Design review of the part built by this model. Coordinates are the model's own, in mm. A direction names the side the tool comes from. Give positions to 0.01 mm unless a question says otherwise; leave off trailing zeros. Order: outer loops, then holes, each group sorted by start corner. A loop starts at its lowest first (then second) coordinate and runs counter-clockwise, first axis right, second up. Notation, with made-up numbers: (-0.75, 56) -> (33.25, 56) arc R9 cw to (33.25, 61) -> close; hole circle Ø8 at (-6, 39.25). An arc over 180 degrees is marked (long way). Use a Markdown table: item, result. Add a question column.
```python
from build123d import *

# Parameters (mm, degrees)
SKETCH_1_W                = 144
SKETCH_1_H                = 35
EXTRUDE_1_DEPTH           = 5
HOLE_WIZARD_1_D           = 4.5
HOLE_WIZARD_1_CSINK_D     = 8.6
HOLE_WIZARD_1_CSINK_ANGLE = 90
SKETCH_4_W                = 100
SKETCH_4_H                = 15
CUT_EXTRUDE_1_DEPTH       = 75.264729179
CHAMFER_1_SIZE            = 3
FILLET_1_R                = 5


with BuildPart() as part:
    # 草图1 → 凸台-拉伸1 (new body)
    with BuildSketch(Plane.XY):
        Rectangle(SKETCH_1_W, SKETCH_1_H)
    extrude(amount=EXTRUDE_1_DEPTH)

    # 打孔尺寸根据十字槽沉头木螺钉的类型1 (through all)
    with Locations(Plane.XY.offset(5)):
        with Locations((-65.75, 7.5), (-65.75, -7.5), (65.75, 7.5), (65.75, -7.5)):
            CounterSinkHole(HOLE_WIZARD_1_D / 2, HOLE_WIZARD_1_CSINK_D / 2, counter_sink_angle=HOLE_WIZARD_1_CSINK_ANGLE)

    # 草图4 → 切除-拉伸1 (cut, through all)
    with BuildSketch(Plane.XY.offset(5)):
        with Locations((0, 10)):
            Rectangle(SKETCH_4_W, SKETCH_4_H)
    extrude(amount=-CUT_EXTRUDE_1_DEPTH, mode=Mode.SUBTRACT)

    # 倒角1
    chamfer_1_edges = [part.edges().sort_by_distance(p)[0] for p in [
        (-50, 17.5, 2.5),
        (50, 17.5, 2.5),
        (72, -17.5, 2.5),
        (-72, -17.5, 2.5),
        (-72, 17.5, 2.5),
        (72, 17.5, 2.5),
    ]]
    chamfer(chamfer_1_edges, length=CHAMFER_1_SIZE)

    # 圆角1
    fillet_1_edges = [part.edges().sort_by_distance(p)[0] for p in [
        (-50, 2.5, 2.5),
        (50, 2.5, 2.5),
    ]]
    fillet(fillet_1_edges, radius=FILLET_1_R)


solid = part.part
```
1) Machinability: for faces 4 (the flat face through (-51.5, 16, 2.5)), 5 (the flat face through (70.5, 16, 2.5)), which of the approach directions +Z, -Z, +X, -X, +Y, -Y give a long, thin tool a straight path to every point of the face, cutting with its end or side? Answer none if there is none.
2) Add section D-D (x = -25). Give the boundary of the cut face in (y, z).
3) Insertion check: pin 1 (2 mm diameter, centred on x = 20.5, z = 4.5, fed in from +Y). The pin has a flat end and moves straight along its axis. Give the tip position at first contact, or say it passes through.
4) Add section C-C (z = 4.1). Give the boundary of the cut face in (x, y).
5) Add section A-A (x = -65.75). Give the boundary of the cut face in (y, z).
6) Add section B-B (y = -7.5). Give the boundary of the cut face in (x, z), then the cut area to 3 significant figures.
7) The part is to be moulded in two halves that separate along X. For faces 1 (the flat face through (70.5, -16, 2.5)), 2 (the flat face through (-50, 11, 3)), 3 (the flat face through (-70.5, -16, 2.5)), say which applies: +X half, -X half, draft (parallel to the pull), parting line (faces both ways), or undercut.
8) For L1, parallel to Y at x = 65.75, z = 1.85; L2, parallel to X at y = 7.5, z = 2.2; L3, parallel to X at y = -7.5, z = 2.25, list the stretches that pass through material, from the lowest coordinate up. Write a range as [from, to].
Worked answers:
| question | item | result |
|---|---|---|
| 1 | face 4 | +Z, -Z, +Y |
| 1 | face 5 | +Z, -Z, +X, +Y |
| 2 | outline | (-17.5, 0) -> (2.5, 0) -> (2.5, 5) -> (-17.5, 5) -> close |
| 3 | pin 1 | y = 2.5 |
| 4 | outline | (-72, -14.5) -> (-69, -17.5) -> (69, -17.5) -> (72, -14.5) -> (72, 14.5) -> (69, 17.5) -> (53, 17.5) -> (50, 14.5) -> (50, 7.5) arc R5 cw to (45, 2.5) -> (-45, 2.5) arc R5 cw to (-50, 7.5) -> (-50, 14.5) -> (-53, 17.5) -> (-69, 17.5) -> (-72, 14.5) -> close; hole circle Ø6.8 at (-65.75, -7.5); hole circle Ø6.8 at (-65.75, 7.5); hole circle Ø6.8 at (65.75, -7.5); hole circle Ø6.8 at (65.75, 7.5) |
| 5 | outline | (-17.5, 0) -> (-9.75, 0) -> (-9.75, 2.95) -> (-11.8, 5) -> (-17.5, 5) -> close; (-5.25, 0) -> (5.25, 0) -> (5.25, 2.95) -> (3.2, 5) -> (-3.2, 5) -> (-5.25, 2.95) -> close; (9.75, 0) -> (17.5, 0) -> (17.5, 5) -> (11.8, 5) -> (9.75, 2.95) -> close |
| 6 | outline | (-72, 0) -> (-68, 0) -> (-68, 2.95) -> (-70.05, 5) -> (-72, 5) -> close; (-63.5, 0) -> (63.5, 0) -> (63.5, 2.95) -> (61.45, 5) -> (-61.45, 5) -> (-63.5, 2.95) -> close; (68, 0) -> (72, 0) -> (72, 5) -> (70.05, 5) -> (68, 2.95) -> close |
| 6 | area | 667 mm^2 |
| 7 | face 1 | +X half |
| 7 | face 2 | undercut |
| 7 | face 3 | -X half |
| 8 | L1 | [-17.5, -9.75], [-5.25, 5.25], [9.75, 17.5] |
| 8 | L2 | [-72, -68], [-63.5, -50], [50, 63.5], [68, 72] |
| 8 | L3 | [-72, -68], [-63.5, 63.5], [68, 72] |
